Geometry: final body of the model. Coordinates: model frame, mm. Face numbers are marked on the shaded views. A direction names the side the tool comes from. Round coordinates to 2 decimals unless told otherwise and drop trailing zeros. Loops run counter-clockwise (first coordinate to the right, second up) from the corner with the lowest first, then second, coordinate; pieces in that order, holes last. Notation, with made-up numbers: (37, 80) -> (81, 80) arc R29 cw to (81, 112) -> close; hole circle Ø4 at (28.25, 31). An arc over 180 degrees is marked (long way). Answer in a Markdown table with one row per item.
```python
from build123d import *

# Parameters (mm, degrees)
BOSS_EXTRUDE1_DEPTH = 5
SKETCH2_W           = 20
SKETCH2_H           = 120
CUT_EXTRUDE1_DEPTH  = 10
CUT_EXTRUDE2_DEPTH  = 140.051478249


with BuildPart() as part:
    # Sketch1 → Boss-Extrude1 (new, symmetric)
    with BuildSketch(Plane.XY):
        with BuildLine():
            Line((-46.360690281, 154.180693982), (-20, 40))
            Line((-20, 40), (-20, 30))
            Line((-20, 30), (0, 30))
            Line((0, 30), (45, 30))
            Line((45, 30), (45, 40))
            Line((45, 40), (45, 154.583310872))
            ThreePointArc((45, 154.583310872), (-0.709503066, 160.998436655), (-46.360690281, 154.180693982))
        make_face()
    extrude(amount=BOSS_EXTRUDE1_DEPTH, both=True)

    # Sketch2 → Cut-Extrude1 (cut)
    with BuildSketch(Plane.XY.offset(5)):
        with Locations((0, 30)):
            Rectangle(SKETCH2_W, SKETCH2_H)
    extrude(amount=-CUT_EXTRUDE1_DEPTH, mode=Mode.SUBTRACT)

    # Sketch3 → Cut-Extrude2 (cut, through all)
    with BuildSketch(Plane.XZ.offset(-30)):
        Polygon((45, -5), (39.904745505, 5), (45, 5), align=None)
    extrude(amount=-CUT_EXTRUDE2_DEPTH, mode=Mode.SUBTRACT)


solid = part.part
```
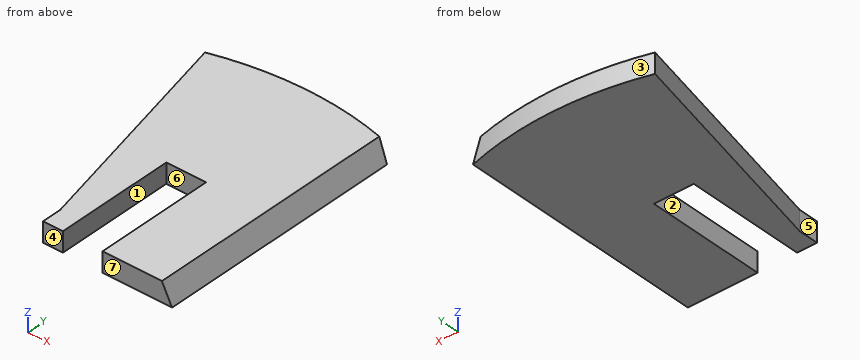
Item 1: Section query A-A, the plane y = 81. Output: boundary loops of the cut face in (x, z).
Ans:
| item | result |
|---|---|
| outline | (-29.47, -5) -> (-10, -5) -> (-10, 5) -> (-29.47, 5) -> close; (10, -5) -> (45, -5) -> (39.9, 5) -> (10, 5) -> close |
Item 2: Set-up query: the marked faces 5, 6 and 7. Return all of +Z, -Z, +X, -X, +Y, -Y with unobstructed straight access to the full face (end or side cutting, diameter ignored); none if empty.
Ans:
| item | result |
|---|---|
| face 5 | +Z, -Z, -X, -Y |
| face 6 | +Z, -Z, -Y |
| face 7 | +Z, -Z, +X, -X, -Y |
Item 3: Section query D-D, the plane y = 130. Output: boundary loops of the cut face in (x, z), and give its area (3 significant figures).
Ans:
| item | result |
|---|---|
| outline | (-40.78, -5) -> (45, -5) -> (39.9, 5) -> (-40.78, 5) -> close |
| area | 832 mm2 |
Item 4: Mould query, pull axis X, two halves, no side actions, for the marked faces 1, 2, 3 and 4. Classes: released by +X, released by -X, zero draft, split by the parting line, or undercut.
Ans:
| item | result |
|---|---|
| face 1 | undercut |
| face 2 | undercut |
| face 3 | split by the parting line |
| face 4 | zero draft |
Item 5: Section query C-C, the plane x = -36.5. Output: boundary loops of the cut face in (y, z).
Ans:
| item | result |
|---|---|
| outline | (111.47, -5) -> (156.81, -5) -> (156.81, 5) -> (111.47, 5) -> close |
Item 6: First-contact query: P1, Ø5, axis at y = 45.5, z = 2.5, coming from the +X side; P2, Ø1.5, axis at x = -9, z = 0, coming from the -Y side; P3, Ø2, axis at x = -2, z = 1.5, coming from the +Y side. Flat tips, straight axial feed; report the tip coordinate or a pass-through.
Ans:
| item | result |
|---|---|
| P1 | x = 42.45 |
| P2 | y = 90 |
| P3 | y = 161 |
Item 7: Ray query, L1, parallel to X at y = 50, z = -3; L2, parallel to X at y = 84, z = 1.75; L3, parallel to Y at x = -1, z = -1.5. Return the intervals inside material, ascending.
Ans:
| item | result |
|---|---|
| L1 | -22.31 to -10, 10 to 43.98 |
| L2 | -30.16 to -10, 10 to 41.56 |
| L3 | 90 to 161 |
Item 8: Section query B-B, the plane z = 2.75. Output: boundary loops of the cut face in (x, y).
Ans:
| item | result |
|---|---|
| outline | (-46.36, 154.18) -> (-20, 40) -> (-20, 30) -> (-10, 30) -> (-10, 90) -> (10, 90) -> (10, 30) -> (41.05, 30) -> (41.05, 155.68) arc R161 ccw to start |
